Job drawing, mm, ordinate dimensions from the low corner. One solid piece. A direction names the side the tool comes from. Round coordinates to 2 decimals unless told otherwise and drop trailing zeros. Loops run counter-clockwise (first coordinate to the right, second up) from the corner with the lowest first, then second, coordinate; pieces in that order, holes last.
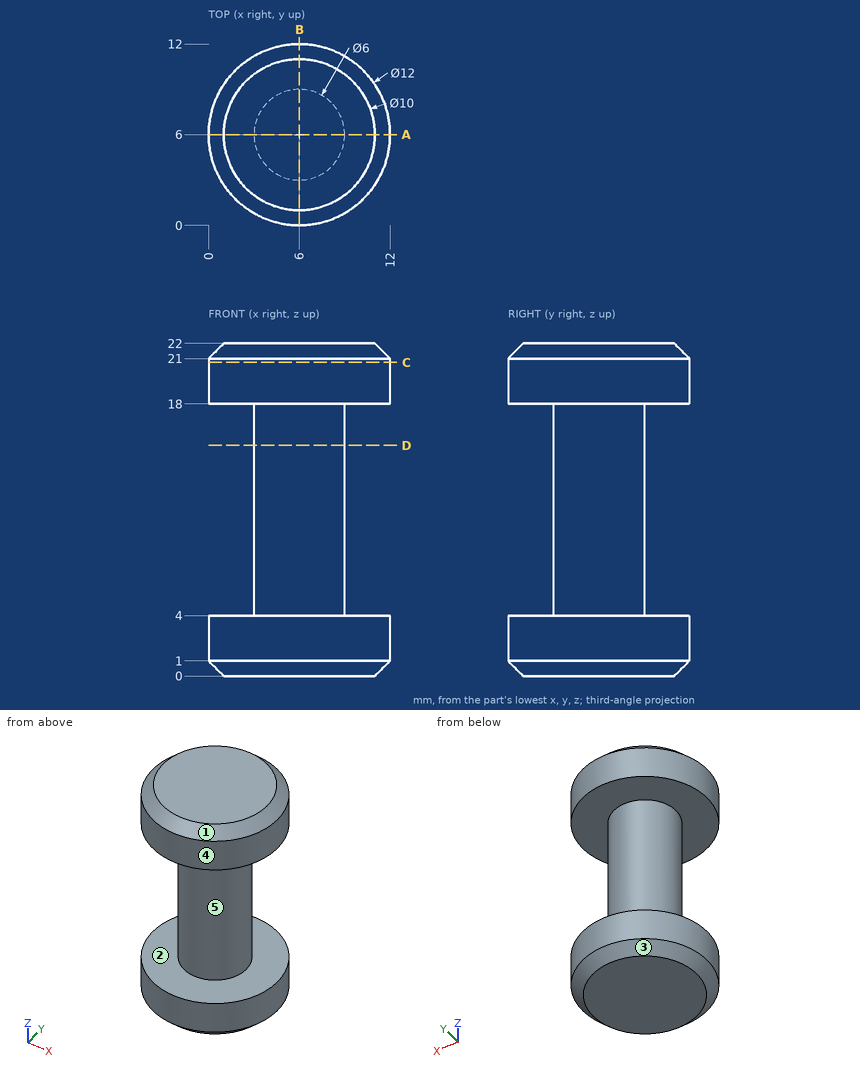
1) Wall check: line 1 along Z through (x, y) = (5.25, 3); line 2 along Z through (x, y) = (7, 0.5); line 3 along X through (y, z) = (4.5, 9.25). Give the ranges that are in metal, low to high.
Values:
line 1: z = 0 to 4, 18 to 22
line 2: z = 0.59 to 4, 18 to 21.41
line 3: x = 3.4 to 8.6
2) Drop flat-ended pins along their axis: pin 1 Ø2 at (x, z) = (9, 18) entering from +Y; pin 2 Ø1 at (y, z) = (2, 3.5) entering from +X. Give the stop position or say it passes through.
Values:
pin 1: stops at y = 11.66
pin 2: stops at x = 10.87
3) Slice it at A-A, the plane y = 6. Give the cut face in (x, z).
Values:
outline: (0, 1) - (1, 0) - (11, 0) - (12, 1) - (12, 4) - (9, 4) - (9, 18) - (12, 18) - (12, 21) - (11, 22) - (1, 22) - (0, 21) - (0, 18) - (3, 18) - (3, 4) - (0, 4) - close
4) Mould opens along Z. For the marked faces 3, 4 and 5 say: released by +Z, released by -Z, zero draft, split by the parting line, or undercut.
Values:
face 3: released by -Z
face 4: zero draft
face 5: undercut
5) Slice it at D-D, the plane z = 15.25. Give the cut face in (x, y).
Values:
outline: circle Ø6 at (6, 6)
6) Tool access for the marked faces 1 and 2: list every direction of +Z, -Z, +X, -X, +Y, -Y with a clear straight run to the whole face (end or side of a thin tool).
Values:
face 1: +Z
face 2: none
7) Slice it at C-C, the plane z = 20.75. Give the cut face in (x, y).
Values:
outline: circle Ø12 at (6, 6)
